Work out the finished part from the listing and answer in its coordinate system (mm). Give positions to 0.01 mm unless a question says otherwise; leave off trailing zeros. Order: outer loops, then holes, each group sorted by start corner. A loop starts at its lowest first (then second) coordinate and runs counter-clockwise, first axis right, second up. Notation, with made-up numbers: (24.5, -32.75) -> (38.5, -32.75) arc R11 ccw to (38.5, -23.75) -> close; hole circle Ø10 at (33, 60.25). An arc over 180 degrees is marked (long way). Use a Markdown table: item, result. Add a question column.
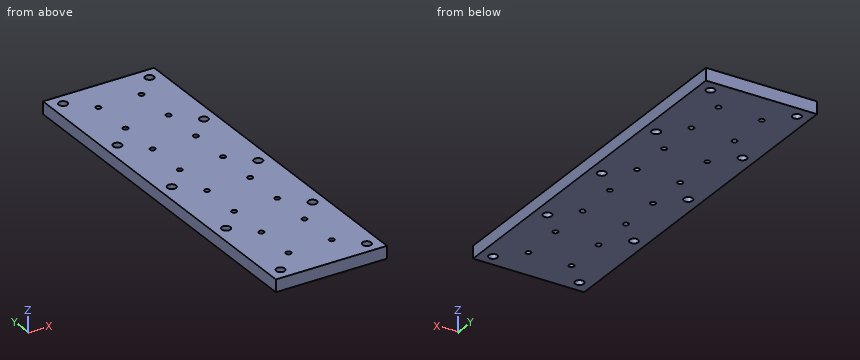
```python
from build123d import *

# Parameters (mm, degrees)
SKETCH1_W                = 90
SKETCH1_H                = 300
BOSS_EXTRUDE1_DEPTH      = 10
F_7_0_7_DIAMETER_HOLE1_D = 7
LPATTERN1_COUNT          = 3
LPATTERN1_PITCH          = 70
LPATTERN1_COUNT_DIR2     = 2
LPATTERN1_PITCH_DIR2     = 70
LPATTERN2_COUNT          = 3
LPATTERN2_PITCH          = 70
LPATTERN2_COPY_1_D       = 7
LPATTERN2_COPY_2_D       = 7
LPATTERN2_COPY_3_D       = 7
LPATTERN2_COPY_4_D       = 7
LPATTERN2_COPY_5_D       = 7
LPATTERN2_COPY_6_D       = 7
LPATTERN2_COPY_7_D       = 7
LPATTERN2_COPY_8_D       = 7
LPATTERN2_COPY_9_D       = 7
LPATTERN2_COPY_10_D      = 7
M5_TAPPED_HOLE1_D        = 4.2
LPATTERN3_COUNT          = 4
LPATTERN3_PITCH          = 35
LPATTERN3_COL_COUNT      = 4
LPATTERN3_COL_PITCH      = 35


with BuildPart() as part:
    # Sketch1 → Boss-Extrude1 (new body)
    with BuildSketch(Plane.XY):
        Rectangle(SKETCH1_W, SKETCH1_H)
    extrude(amount=BOSS_EXTRUDE1_DEPTH)

    # Ø7.0 (7) Diameter Hole1 (through all)
    with Locations(Plane.XY.offset(10)):
        with Locations((-35, 0)):
            f_7_0_7_diameter_hole1 = Hole(F_7_0_7_DIAMETER_HOLE1_D / 2)

    # LPattern1: 7.0 _7_ Diameter Hole1 3 × 2
    with Locations(*[(j * LPATTERN1_PITCH_DIR2, -i * LPATTERN1_PITCH, 0) for i in range(LPATTERN1_COUNT) for j in range(LPATTERN1_COUNT_DIR2) if (i, j) != (0, 0)]):
        add(f_7_0_7_diameter_hole1, mode=Mode.SUBTRACT)

    # LPattern2: Ø7.0 (7) Diameter Hole1 ×3
    with Locations(*[(0, i * LPATTERN2_PITCH, 0) for i in range(1, LPATTERN2_COUNT)]):
        add(f_7_0_7_diameter_hole1, mode=Mode.SUBTRACT)

    # LPattern2 copy 1 (through all)
    with Locations(Plane(origin=(70, 70, 10), x_dir=(1, 0, 0), z_dir=(0, 0, 1))):
        with Locations((-35, 0)):
            Hole(LPATTERN2_COPY_1_D / 2)

    # LPattern2 copy 2 (through all)
    with Locations(Plane(origin=(70, 140, 10), x_dir=(1, 0, 0), z_dir=(0, 0, 1))):
        with Locations((-35, 0)):
            Hole(LPATTERN2_COPY_2_D / 2)

    # LPattern2 copy 3 (through all)
    with Locations(Plane.XY.offset(10)):
        with Locations((-35, 0)):
            Hole(LPATTERN2_COPY_3_D / 2)

    # LPattern2 copy 4 (through all)
    with Locations(Plane(origin=(0, 70, 10), x_dir=(1, 0, 0), z_dir=(0, 0, 1))):
        with Locations((-35, 0)):
            Hole(LPATTERN2_COPY_4_D / 2)

    # LPattern2 copy 5 (through all)
    with Locations(Plane(origin=(70, 0, 10), x_dir=(1, 0, 0), z_dir=(0, 0, 1))):
        with Locations((-35, 0)):
            Hole(LPATTERN2_COPY_5_D / 2)

    # LPattern2 copy 6 (through all)
    with Locations(Plane(origin=(70, 70, 10), x_dir=(1, 0, 0), z_dir=(0, 0, 1))):
        with Locations((-35, 0)):
            Hole(LPATTERN2_COPY_6_D / 2)

    # LPattern2 copy 7 (through all)
    with Locations(Plane(origin=(0, -70, 10), x_dir=(1, 0, 0), z_dir=(0, 0, 1))):
        with Locations((-35, 0)):
            Hole(LPATTERN2_COPY_7_D / 2)

    # LPattern2 copy 8 (through all)
    with Locations(Plane.XY.offset(10)):
        with Locations((-35, 0)):
            Hole(LPATTERN2_COPY_8_D / 2)

    # LPattern2 copy 9 (through all)
    with Locations(Plane(origin=(70, -70, 10), x_dir=(1, 0, 0), z_dir=(0, 0, 1))):
        with Locations((-35, 0)):
            Hole(LPATTERN2_COPY_9_D / 2)

    # LPattern2 copy 10 (through all)
    with Locations(Plane(origin=(70, 0, 10), x_dir=(1, 0, 0), z_dir=(0, 0, 1))):
        with Locations((-35, 0)):
            Hole(LPATTERN2_COPY_10_D / 2)

    # M5 Tapped Hole1 (through all)
    with Locations(Plane(origin=(0, 0, 0), x_dir=(-1, 0, 0), z_dir=(0, 0, -1))):
        with Locations((17.5, 17.5), (17.5, -17.5), (-17.5, -17.5), (-17.5, 17.5)):
            m5_tapped_hole1 = Hole(M5_TAPPED_HOLE1_D / 2)

    # LPattern3: M5 Tapped Hole1 ×4
    with Locations(*[(0, -i * LPATTERN3_PITCH, 0) for i in range(1, LPATTERN3_COUNT)]):
        add(m5_tapped_hole1, mode=Mode.SUBTRACT)

    # LPattern3 col: M5 Tapped Hole1 ×4
    with Locations(*[(0, i * LPATTERN3_COL_PITCH, 0) for i in range(1, LPATTERN3_COL_COUNT)]):
        add(m5_tapped_hole1, mode=Mode.SUBTRACT)


solid = part.part
```
1) A flat-ended cylindrical pin translates along its axis: pin 1 (4 mm diameter, centred on x = 17.5, y = -17.5, fed in from +Z). Find the tip coordinate at first contact, or state that the pin passes through.
2) The part is cut by section B-B, the plane z = 5.5. State how many separate pieces and enclosed holes the cut face has, then the cut area to 3 significant figures.
3) The part is cut by section A-A, the plane y = 70. Determine the outline of the cut face in (x, z).
4) Straight lines are drawn through the part: line 1 (Y direction, x = -35, z = 5); line 2 (X direction, y = -140, z = 4.25); line 3 (Y direction, x = 37.5, z = 6). For each, find the intervals that lie inside material, in ascending order.
A:
| question | item | result |
|---|---|---|
| 1 | pin 1 | through |
| 2 | separate pieces | 1 |
| 2 | enclosed holes | 26 |
| 2 | area | 26,400 mm^2 |
| 3 | outline | (-45, 0) -> (-38.5, 0) -> (-38.5, 10) -> (-45, 10) -> close; (-31.5, 0) -> (31.5, 0) -> (31.5, 10) -> (-31.5, 10) -> close; (38.5, 0) -> (45, 0) -> (45, 10) -> (38.5, 10) -> close |
| 4 | line 1 | -150 to -143.5, -136.5 to -73.5, -66.5 to -3.5, 3.5 to 66.5, 73.5 to 136.5, 143.5 to 150 |
| 4 | line 2 | -45 to -38.5, -31.5 to 31.5, 38.5 to 45 |
| 4 | line 3 | -150 to -142.45, -137.55 to -72.45, -67.55 to -2.45, 2.45 to 67.55, 72.45 to 137.55, 142.45 to 150 |
